from build123d import *

# Parameters (mm, degrees)
SQUARE_TUBE_40_X_40_X_4_1_DEPTH = 870


with BuildPart() as part:
    # Sketch1 → Square Tube 40 X 40 X 4(1) (new body)
    with BuildSketch(Plane.YZ.offset(-1000)):
        with BuildLine():
            Line((-12, -20), (12, -20))
            ThreePointArc((12, -20), (17.656854249, -17.656854249), (20, -12))
            Line((20, -12), (20, 12))
            ThreePointArc((20, 12), (17.656854249, 17.656854249), (12, 20))
            Line((12, 20), (-12, 20))
            ThreePointArc((-12, 20), (-17.656854249, 17.656854249), (-20, 12))
            Line((-20, 12), (-20, -12))
            ThreePointArc((-20, -12), (-17.656854249, -17.656854249), (-12, -20))
        make_face()
        with BuildLine():
            Line((-12, -16), (12, -16))
            ThreePointArc((12, -16), (14.828427125, -14.828427125), (16, -12))
            Line((16, -12), (16, 12))
            ThreePointArc((16, 12), (14.828427125, 14.828427125), (12, 16))
            Line((12, 16), (-12, 16))
            ThreePointArc((-12, 16), (-14.828427125, 14.828427125), (-16, 12))
            Line((-16, 12), (-16, -12))
            ThreePointArc((-16, -12), (-14.828427125, -14.828427125), (-12, -16))
        make_face(mode=Mode.SUBTRACT)
    extrude(amount=SQUARE_TUBE_40_X_40_X_4_1_DEPTH)


solid = part.part
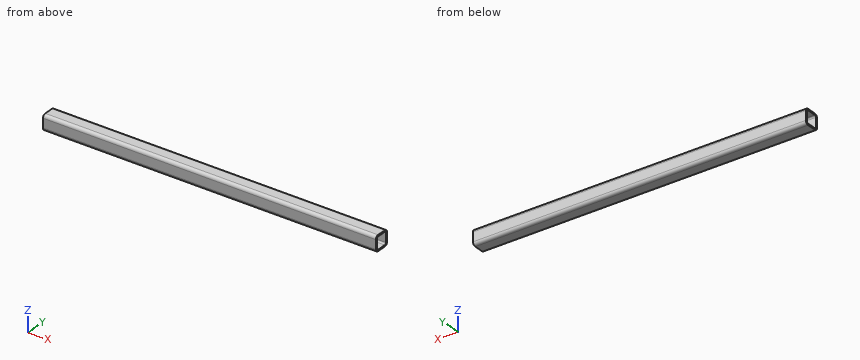
Geometry check sheet. Reference: the model listing, model coordinates, mm. Round coordinates to 2 decimals unless told otherwise and drop trailing zeros. Order: outer loops, then holes, each group sorted by start corner. A loop starts at its lowest first (then second) coordinate and runs counter-clockwise, first axis right, second up. Notation, with made-up numbers: M 27,72 L 84,72 A31 ccw 84,106 Z; hole C 13.5,49 d3. An arc over 180 degrees is marked long. Write each question's results on one line, items separated by ' | '. Start each with the question number.
1. Cross-section at C-C on x = -396.5. Record the boundary of the cut face in (y, z), plus the area to 3 significant figures.
2. Material ranges on L1, parallel to Y at x = -446, z = 6.5; L2, parallel to Y at x = -870, z = -14.5, recorded low to high. Write a range as from..to.
3. Cross-section at A-A on y = 2.5. Record the boundary of the cut face in (x, z), plus the area to 3 significant figures.
Resolved:
1) outline: M -20,-12 A8 ccw -12,-20 L 12,-20 A8 ccw 20,-12 L 20,12 A8 ccw 12,20 L -12,20 A8 ccw -20,12 Z; hole M -16,-12 A4 ccw -12,-16 L 12,-16 A4 ccw 16,-12 L 16,12 A4 ccw 12,16 L -12,16 A4 ccw -16,12 Z | area: 535 mm2
2) L1: -20..-16, 16..20 | L2: -19.6..-15.12, 15.12..19.6
3) outline: M -1000,-20 L -130,-20 L -130,-16 L -1000,-16 Z; M -1000,16 L -130,16 L -130,20 L -1000,20 Z | area: 6,960 mm2
